Read the model definition and answer for the solid it produces. Units are mm, in the model's axes. A direction names the side the tool comes from. Give positions to 0.01 mm unless a question says otherwise; leave off trailing zeros. Order: outer loops, then holes, each group sorted by start corner. A loop starts at its lowest first (then second) coordinate and runs counter-clockwise, first axis right, second up. Notation, with made-up numbers: (-26.75, 85) - (13.25, 85) arc R11 cw to (13.25, 97) - close; hole circle Ø6 at (56.25, 33.5). An arc over 180 degrees is marked (long way). Use a Markdown table: item, result. Add a question column.
1. A cutting plane is placed at C-C on z = 51. Determine the outline of the cut face in (x, y).
2. A cutting plane is placed at A-A on y = -7. Determine the outline of the cut face in (x, z), and give its area (3 significant figures).
3. Which of the six approach directions +Z, -Z, +X, -X, +Y, -Y give full straight-line access (tool end or side, diameter ignored) to faces 5 (the flat face through (-25, 0, 1)), 6 (the flat face through (0, 22, 1))?
4. Consider L1, parallel to Y at x = 14, z = 30.5; L2, parallel to Y at x = 20, z = -41. Determine where each line is inside the solid, lowest interval first.
5. For a pull along Y with two mould halves and no side action, classify faces 1 (the flat face through (0.1, -22.3, 87.5)), 2 (the flat face through (0, 25, 1)), 3 (the cylindrical face through (21.14, -21.1, 1.22)), 4 (the cylindrical face through (23.289, -23.196, 1.225)) as released by +Y, released by -Y, zero draft, split by the parting line, or undercut.
```python
from build123d import *

# Parameters (mm, degrees)
GB_6728_1986_050_X_50_X_3_1_DEPTH = 175


with BuildPart() as part:
    # Sketch1 → Gb／6728-1986方形空心型钢 050 X 50 X 3(1) (new body)
    with BuildSketch(Plane.YX.offset(-87.5)):
        with BuildLine():
            Line((-19, -25), (19, -25))
            ThreePointArc((19, -25), (23.242640687, -23.242640687), (25, -19))
            Line((25, -19), (25, 19))
            ThreePointArc((25, 19), (23.242640687, 23.242640687), (19, 25))
            Line((19, 25), (-19, 25))
            ThreePointArc((-19, 25), (-23.242640687, 23.242640687), (-25, 19))
            Line((-25, 19), (-25, -19))
            ThreePointArc((-25, -19), (-23.242640687, -23.242640687), (-19, -25))
        make_face()
        with BuildLine():
            Line((-19, -22), (19, -22))
            ThreePointArc((19, -22), (21.121320344, -21.121320344), (22, -19))
            Line((22, -19), (22, 19))
            ThreePointArc((22, 19), (21.121320344, 21.121320344), (19, 22))
            Line((19, 22), (-19, 22))
            ThreePointArc((-19, 22), (-21.121320344, 21.121320344), (-22, 19))
            Line((-22, 19), (-22, -19))
            ThreePointArc((-22, -19), (-21.121320344, -21.121320344), (-19, -22))
        make_face(mode=Mode.SUBTRACT)
    extrude(amount=GB_6728_1986_050_X_50_X_3_1_DEPTH)


solid = part.part
```
Output values:
| question | item | result |
|---|---|---|
| 1 | outline | (-25, -19) arc R6 ccw to (-19, -25) - (19, -25) arc R6 ccw to (25, -19) - (25, 19) arc R6 ccw to (19, 25) - (-19, 25) arc R6 ccw to (-25, 19) - close; hole (-22, -19) arc R3 ccw to (-19, -22) - (19, -22) arc R3 ccw to (22, -19) - (22, 19) arc R3 ccw to (19, 22) - (-19, 22) arc R3 ccw to (-22, 19) - close |
| 2 | outline | (-25, -87.5) - (-22, -87.5) - (-22, 87.5) - (-25, 87.5) - close; (22, -87.5) - (25, -87.5) - (25, 87.5) - (22, 87.5) - close |
| 2 | area | 1,050 mm² |
| 3 | face 5 | +Z, -Z, -X, +Y, -Y |
| 3 | face 6 | +Z, -Z |
| 4 | L1 | -25 to -22, 22 to 25 |
| 4 | L2 | -24.92 to -21.83, 21.83 to 24.92 |
| 5 | face 1 | zero draft |
| 5 | face 2 | released by +Y |
| 5 | face 3 | undercut |
| 5 | face 4 | released by -Y |
